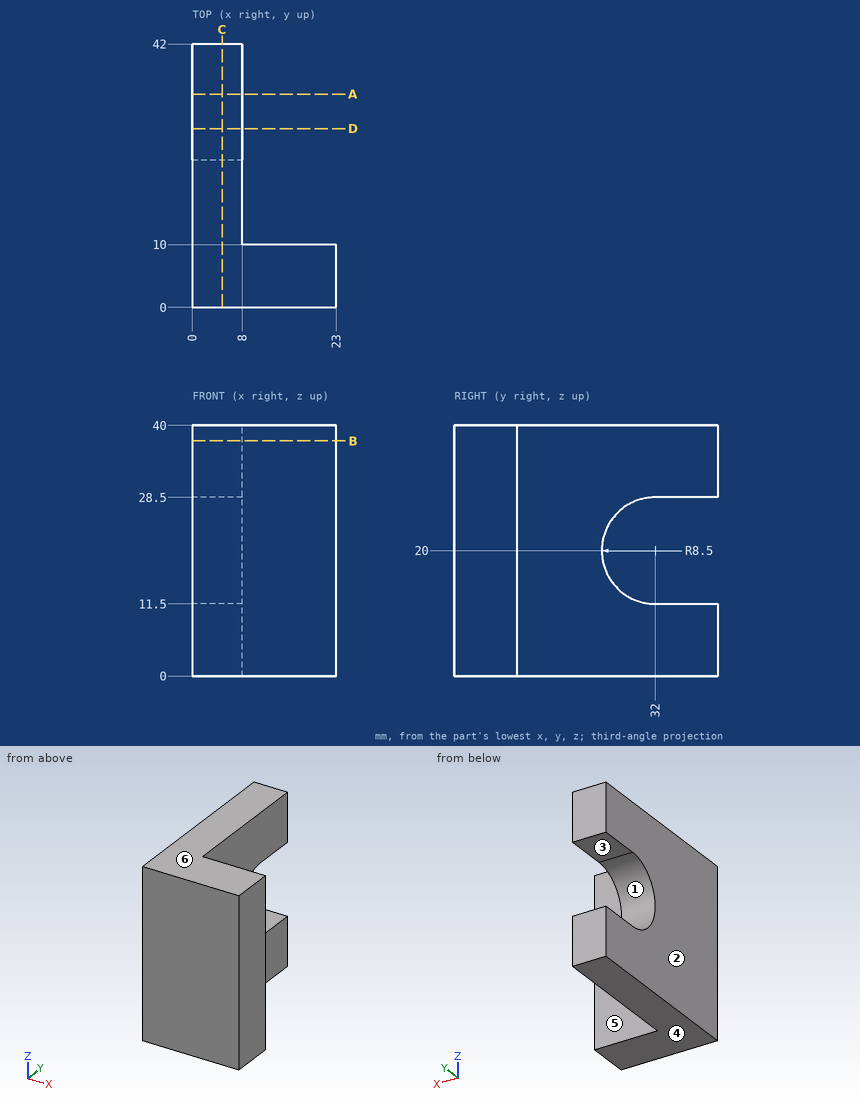
Answer from the drawing. Dimensions are ordinates in mm from the lowest x, y and z of the part. A direction names the side the tool comes from. Round coordinates to 2 decimals unless told otherwise and drop trailing zeros. Loops run counter-clockwise (first coordinate to the right, second up) from the corner with the lowest first, then second, coordinate; pieces in that order, holes last. Notation, with made-up numbers: M 67,-12 L 86,-12 A16 cw 86,5 Z; hole C -2,-0.5 d8. An arc over 180 degrees is marked long. One line per question, with ' | ' between items. Start each with the question number.
(1) A cutting plane is placed at A-A on y = 34. Write down the section's boundary in (x, z), plus the area to 3 significant figures.
(2) A cutting plane is placed at D-D on y = 28.5. Write down the section's boundary in (x, z), plus the area to 3 significant figures.
(3) A cutting plane is placed at C-C on x = 4.75. Write down the section's boundary in (y, z).
(4) A cutting plane is placed at B-B on z = 37.5. Write down the section's boundary in (x, y), plus the area to 3 significant figures.
(5) Find the intervals of material crossed by line 1 (Y direction, x = 13.25, z = 22); line 2 (X direction, y = 18, z = 19); line 3 (Y direction, x = 1.25, z = 27), in increasing order.
(6) A flat-ended cylindrical pin translates along its axis: pin 1 Ø12 at (x, z) = (12.5, 28) entering from +Y. Find the tip coordinate at first contact, or state that the pin passes through.
(7) For a pull along Z with two mould halves and no side action, classify the marked faces 1, 2, 3 and 4 as released by +Z, released by -Z, zero draft, split by the parting line, or undercut.
(8) A tool of negligible diameter and unlimited length cuts with its end or side. For the marked faces 5 and 6, from which of +Z, -Z, +X, -X, +Y, -Y can it reach the whole face along a straight path? Write none if from no direction.
Geometry check:
1) outline: M 0,0 L 8,0 L 8,11.5 L 0,11.5 Z; M 0,28.5 L 8,28.5 L 8,40 L 0,40 Z | area: 184 mm²
2) outline: M 0,0 L 8,0 L 8,12.25 L 0,12.25 Z; M 0,27.75 L 8,27.75 L 8,40 L 0,40 Z | area: 196 mm²
3) outline: M 0,0 L 42,0 L 42,11.5 L 32,11.5 A8.5 cw 32,28.5 L 42,28.5 L 42,40 L 0,40 Z
4) outline: M 0,0 L 23,0 L 23,10 L 8,10 L 8,42 L 0,42 Z | area: 486 mm²
5) line 1: y = 0 to 10 | line 2: x = 0 to 8 | line 3: y = 0 to 27.18
6) pin 1: stops at y = 42
7) face 1: undercut | face 2: zero draft | face 3: undercut | face 4: released by -Z
8) face 5: +Z, -Z, +X, +Y | face 6: +Z, +X, -X, +Y, -Y
